from build123d import *

# Parameters (mm, degrees)
SKETCH1_W           = 40
SKETCH1_H           = 40
BOSS_EXTRUDE1_DEPTH = 15
CHAMFER1_SIZE       = 4
BOSS_EXTRUDE2_DEPTH = 5
SKETCH4_R           = 10
BOSS_EXTRUDE3_DEPTH = 2
SKETCH5_R           = 2.5
BOSS_EXTRUDE4_DEPTH = 22
CUT_EXTRUDE1_START  = -2
SKETCH6_R           = 4
SKETCH6_R_2         = 2.5
CUT_EXTRUDE1_DEPTH  = 2
CHAMFER2_SIZE       = 0.5
SKETCH7_R           = 2
CUT_EXTRUDE2_DEPTH  = 49.989794856


with BuildPart() as part:
    # Sketch1 → Boss-Extrude1 (new, symmetric)
    with BuildSketch(Plane.XY):
        Rectangle(SKETCH1_W, SKETCH1_H)
    extrude(amount=BOSS_EXTRUDE1_DEPTH, both=True)

    # Chamfer1
    chamfer1_edges = [part.edges().sort_by_distance(p)[0] for p in [
        (-20, 20, 0),
        (20, 20, 0),
        (20, -20, 0),
        (-20, -20, 0),
    ]]
    chamfer(chamfer1_edges, length=CHAMFER1_SIZE)

    # Sketch3 → Boss-Extrude2 (add)
    with BuildSketch(Plane.XY.offset(15)):
        Polygon((15, -20), (-15, -20), (-20, -15), (-20, 15), (-15, 20), (17, 20), (20, 17), (20, -15), align=None)
    boss_extrude2 = extrude(amount=BOSS_EXTRUDE2_DEPTH)

    # Mirror1: Boss-Extrude2 across plane
    add(boss_extrude2.mirror(Plane.XY))

    # Sketch4 → Boss-Extrude3 (add)
    with BuildSketch(Plane.XY.offset(20)):
        with Locations(Location((0, 0, 0), (0, 0, 180))):
            Circle(SKETCH4_R)
    extrude(amount=BOSS_EXTRUDE3_DEPTH)

    # Sketch5 → Boss-Extrude4 (add)
    with BuildSketch(Plane.XY.offset(22)):
        Circle(SKETCH5_R)
    extrude(amount=BOSS_EXTRUDE4_DEPTH)

    # Sketch6 → Cut-Extrude1 (cut)
    with BuildSketch(Plane.XY.offset(22).offset(CUT_EXTRUDE1_START)):
        Circle(SKETCH6_R)
        Circle(SKETCH6_R_2, mode=Mode.SUBTRACT)
    extrude(amount=CUT_EXTRUDE1_DEPTH, mode=Mode.SUBTRACT)

    # Chamfer2
    chamfer2_edges = [part.edges().sort_by_distance(p)[0] for p in [
        (-2.5, 0, 44),
    ]]
    chamfer(chamfer2_edges, length=CHAMFER2_SIZE)

    # Sketch7 → Cut-Extrude2 (cut, through all)
    with BuildSketch(Plane.XY.offset(20)):
        with Locations((16, 16)):
            Circle(SKETCH7_R)
        with Locations((16, -16)):
            Circle(SKETCH7_R)
        with Locations((-16, -16)):
            Circle(SKETCH7_R)
        with Locations((-16, 16)):
            Circle(SKETCH7_R)
    extrude(amount=-CUT_EXTRUDE2_DEPTH, mode=Mode.SUBTRACT)


solid = part.part
Build history of the part. All positions in model axes, mm. A direction names the side the tool comes from. Coordinates: 2 decimals unless noted, no trailing zeros. Order: outer loops, then holes, each group sorted by start corner. A loop starts at its lowest first (then second) coordinate and runs counter-clockwise, first axis right, second up. Notation, with made-up numbers: (-17, 48.5) -> (27, 48.5) arc R9 cw to (27, 60.5) -> close; hole circle Ø2 at (16.25, -2). An arc over 180 degrees is marked (long way). One line per item, written item: value.
(1) Drop a flat-ended pin along its axis: pin 1 Ø10 at (x, y) = (-5, 15.5) entering from +Z. Give the stop position or say it passes through.
Checked values:
pin 1: z = 20
(2) Slice it at B-B, the plane y = -6. List the corners of the cut face in (x, z).
Checked values:
outline: (-20, -20) -> (20, -20) -> (20, 20) -> (8, 20) -> (8, 22) -> (-8, 22) -> (-8, 20) -> (-20, 20) -> close
(3) Tool access for faces 5 (the flat face through (18, -17, 17)), 6 (the flat face through (-18, 17, -17)), 7 (the cylindrical face through (-0.54, -2.44, 31.59)): list every direction of +Z, -Z, +X, -X, +Y, -Y with a clear straight run to the whole face (end or side of a thin tool).
Checked values:
face 5: +Z, +X, -Y
face 6: -Z, -X, +Y
face 7: +Z
(4) Mould opens along X. For faces 1 (the cylindrical face through (10, 0, 21)), 2 (the cylindrical face through (16, -14, 0)), 3 (the flat face through (18, -17, -17)), 4 (the flat face through (0, 0, 44)) say: pulls with the +X half, pulls with the -X half, needs draft (parallel to the pull), parting line crosses it, or undercut.
Checked values:
face 1: parting line crosses it
face 2: undercut
face 3: pulls with the +X half
face 4: needs draft
(5) Slice it at A-A, the plane z = 16.5. List the corners of the cut face in (x, y).
Checked values:
outline: (-20, -15) -> (-15, -20) -> (15, -20) -> (20, -15) -> (20, 17) -> (17, 20) -> (-15, 20) -> (-20, 15) -> close; hole circle Ø4 at (-16, -16); hole circle Ø4 at (-16, 16); hole circle Ø4 at (16, -16); hole circle Ø4 at (16, 16)
(6) Slice it at C-C, the plane x = 0. List the corners of the cut face in (y, z).
Checked values:
outline: (-20, -20) -> (20, -20) -> (20, 20) -> (10, 20) -> (10, 22) -> (4, 22) -> (4, 20) -> (2.5, 20) -> (2.5, 43.5) -> (2, 44) -> (-2, 44) -> (-2.5, 43.5) -> (-2.5, 20) -> (-4, 20) -> (-4, 22) -> (-10, 22) -> (-10, 20) -> (-20, 20) -> close
(7) Probe line 1 (Y direction, x = 0, z = 20.95); line 2 (Y direction, x = -16, z = 9); line 3 (Z direction, x = 14, y = 12). List the from-to ranges inside material, lowest first. Write a range as [from, to].
Checked values:
line 1: [-10, -4], [-2.5, 2.5], [4, 10]
line 2: [-20, -18], [-14, 14], [18, 20]
line 3: [-20, 20]
(8) Slice it at D-D, the plane z = -12.5. List the corners of the cut face in (x, y), plus the area to 3 significant figures.
Checked values:
outline: (-20, -16) -> (-16, -20) -> (16, -20) -> (20, -16) -> (20, 16) -> (16, 20) -> (-16, 20) -> (-20, 16) -> close; hole circle Ø4 at (-16, -16); hole circle Ø4 at (-16, 16); hole circle Ø4 at (16, -16); hole circle Ø4 at (16, 16)
area: 1,520 mm2
